Build history of the part. All positions in model axes, mm. Round coordinates to 2 decimals unless told otherwise and drop trailing zeros. Write each loop counter-clockwise with the first axis right and the second up, starting at its lowest first coordinate (ties: lowest second). Pieces come first, ordered by that corner, then holes. Notation, with made-up numbers: (7.25, -7) -> (24.25, -7) arc R24 cw to (24.25, 21) -> close; hole circle Ø8 at (-4, 68.25). An arc over 180 degrees is marked (long way). Return JSON: item names as keys, results as strings.
from build123d import *

# Parameters (mm, degrees)
EXTRUDE_1_DEPTH    = 575
HOLE_WIZARD_M6_1_D = 5


with BuildPart() as part:
    # 草图1 → 凸台-拉伸1 (new body)
    with BuildSketch(Plane.XY):
        with BuildLine():
            Line((0, 0), (-45, 0))
            Line((-45, 0), (-45, -80))
            Line((-45, -80), (0, -80))
            Line((0, -80), (0, -78.639315732))
            ThreePointArc((0, -78.639315732), (-0.981161679, -76.015079616), (-3.443307596, -74.678243457))
            Line((-3.443307596, -74.678243457), (-32.113384808, -70.648926875))
            ThreePointArc((-32.113384808, -70.648926875), (-37.037676642, -67.975254557), (-39, -62.726782325))
            Line((-39, -62.726782325), (-39, -17.273217675))
            ThreePointArc((-39, -17.273217675), (-37.037676642, -12.024745443), (-32.113384808, -9.351073125))
            Line((-32.113384808, -9.351073125), (-3.443307596, -5.321756543))
            ThreePointArc((-3.443307596, -5.321756543), (-0.981161679, -3.984920384), (0, -1.360684268))
            Line((0, -1.360684268), (0, 0))
        make_face()
    extrude(amount=EXTRUDE_1_DEPTH)

    # M6 螺纹孔1 (through all)
    with Locations(Plane(origin=(0, -80, 0), x_dir=(-1, 0, 0), z_dir=(0, -1, 0))):
        with Locations((22.5, -445)):
            Hole(HOLE_WIZARD_M6_1_D / 2)


solid = part.part
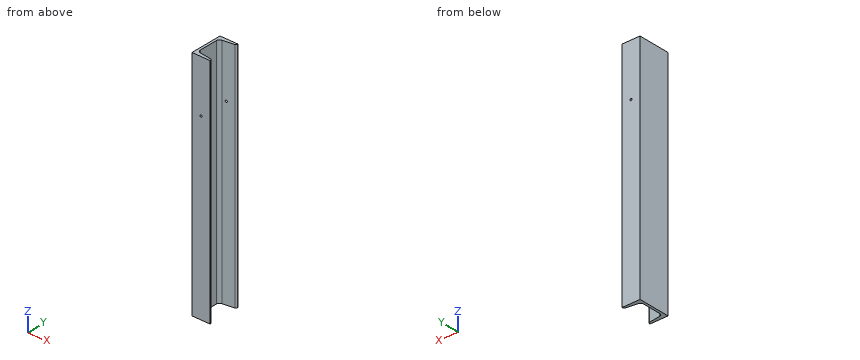
Q1. Saw through at C-C on y = -47. List the corners of the cut face in (x, z), then the cut area to 3 significant figures.
Verdict:
{"outline": "(-45, 0) -> (-39, 0) -> (-39, 575) -> (-45, 575) -> close", "area": "3,450 mm²"}
Q2. Saw through at A-A on z = 353. List the corners of the cut face in (x, y), then the cut area to 3 significant figures.
Verdict:
{"outline": "(-45, -80) -> (0, -80) -> (0, -78.64) arc R4 ccw to (-3.44, -74.68) -> (-32.11, -70.65) arc R8 cw to (-39, -62.73) -> (-39, -17.27) arc R8 cw to (-32.11, -9.35) -> (-3.44, -5.32) arc R4 ccw to (0, -1.36) -> (0, 0) -> (-45, 0) -> close", "area": "1,090 mm²"}
Q3. Saw through at B-B on x = -12.5. List the corners of the cut face in (y, z).
Verdict:
{"outline": "(-80, 0) -> (-73.41, 0) -> (-73.41, 575) -> (-80, 575) -> close; (-6.59, 0) -> (0, 0) -> (0, 575) -> (-6.59, 575) -> close"}
Q4. Pin check, flat tips, straight feed: pin 1 Ø12 at (y, z) = (-42.5, 85.5) entering from +X; pin 2 Ø10 at (y, z) = (-19.5, 189) entering from +X. Stop position of each tip, or through.
Verdict:
{"pin 1": "stops at x = -39", "pin 2": "stops at x = -38.5"}
Q5. Wall check: L1, parallel to Z at x = -22, y = -5; L2, parallel to Z at x = -22.5, y = -75.25; L3, parallel to X at y = -37.5, z = 392.5. Give the ranges that are in metal, low to high.
Verdict:
{"L1": "z = 0 to 442.55, 447.45 to 575", "L2": "z = 0 to 442.5, 447.5 to 575", "L3": "x = -45 to -39"}
